Build history of the part. All positions in model axes, mm. A direction names the side the tool comes from. Coordinates: 2 decimals unless noted, no trailing zeros. Loops run counter-clockwise (first coordinate to the right, second up) from the corner with the lowest first, then second, coordinate; pieces in that order, holes last.
Item 1: Cut at C-C (x = -2.5). List the corners of the cut face in (y, z), and give its area (3 significant figures).
Item 2: 3-axis set-ups, long thin cutter, end or side, ignore diameter. For faces 1 (the face through (27.59, 1.05, 3.91)), 2 (the face through (0, -7.6, 11)), 3 (the face through (0, 7.6, 11)), 4 (the face through (0, 18, 2)), 5 (the face through (-10.336, -11.567, 1.724)): which of +Z, -Z, +X, -X, +Y, -Y reach the whole face in a straight line?
Item 3: Mould opens along X. For faces 6 (the face through (18.85, 0.17, 10.63)), 7 (the face through (0, -18, 2)), 8 (the face through (-29.246, -0.396, 2.169)), 9 (the face through (12.87, 13.51, 1.72)) say: released by +X, released by -X, zero draft, split by the parting line, or undercut.
Item 4: Drill centre lines: line 1 along Y through (x, z) = (11.25, 1.6); line 2 along X through (y, z) = (2, 5.5); line 3 along Z through (x, y) = (-19.5, 6). Where is each one in solid material? Low to high.
Item 5: Cut at A-A (z = 14). List the corners of the cut face in (x, y), and give its area (3 significant figures).
Item 6: Cut at D-D (y = -13). List the corners of the cut face in (x, z), and give its area (3 significant figures).
Item 7: Flat gauge pins, fed straight in: pin 1 (1 mm diameter, centred on x = -16, z = 14, fed in from -Y); pin 2 (8 mm diameter, centred on x = 4.5, y = -8, fed in from -Z); pin 3 (5.5 mm diameter, centred on x = 22.5, y = 0.5, fed in from +Z); pin 4 (8 mm diameter, centred on y = -8, z = 3.5, fed in from +X). Where does each tip first touch, or does it go through?
Item 8: Cut at B-B (x = 24.25). List the corners of the cut face in (y, z), and give its area (3 significant figures).
from build123d import *

# Parameters (mm, degrees)
OVAL_BASE_FLANGE_DEPTH       = 4.4
RAISED_OBROUND_HOUSING_DEPTH = 11.6
HOUSING_SLOT_R5_DEPTH        = 5
MOUNTING_HOLES_SKETCH_R      = 1.7
MOUNTING_HOLES_6X_3_4_DEPTH  = 5
COUNTERBORE_SKETCH_R         = 3.5
COUNTERBORES_6X_7_DEPTH      = 1
SLOT_THROUGH_CUT_SKETCH_R    = 2.5
SLOT_THROUGH_CUT_DEPTH       = 37.063312383
HOUSING_BASE_FILLET_R1_R     = 1


with BuildPart() as part:
    # Flange Profile Sketch → Oval Base Flange (new body)
    with BuildSketch(Plane.XY):
        with BuildLine():
            Line((-11.25, 18), (11.25, 18))
            ThreePointArc((11.25, 18), (29.25, 0), (11.25, -18))
            Line((11.25, -18), (-11.25, -18))
            ThreePointArc((-11.25, -18), (-29.25, 0), (-11.25, 18))
        make_face()
    extrude(amount=OVAL_BASE_FLANGE_DEPTH)

    # Housing Profile Sketch → Raised Obround Housing (add)
    with BuildSketch(Plane.XY.offset(4.4)):
        with BuildLine():
            Line((-11.25, 7.6), (11.25, 7.6))
            ThreePointArc((11.25, 7.6), (18.85, 0), (11.25, -7.6))
            Line((11.25, -7.6), (-11.25, -7.6))
            ThreePointArc((-11.25, -7.6), (-18.85, 0), (-11.25, 7.6))
        make_face()
    extrude(amount=RAISED_OBROUND_HOUSING_DEPTH)

    # Housing Slot Sketch → Housing Slot R5 (cut)
    with BuildSketch(Plane.XY.offset(16)):
        with BuildLine():
            Line((-11.25, 5), (11.25, 5))
            ThreePointArc((11.25, 5), (16.25, 0), (11.25, -5))
            Line((11.25, -5), (-11.25, -5))
            ThreePointArc((-11.25, -5), (-16.25, 0), (-11.25, 5))
        make_face()
    extrude(amount=-HOUSING_SLOT_R5_DEPTH, mode=Mode.SUBTRACT)

    # Mounting Holes Sketch → Mounting Holes 6xØ3.4 (cut)
    with BuildSketch(Plane.XY.offset(4.4)):
        with Locations((-24.22204296, 0)):
            Circle(MOUNTING_HOLES_SKETCH_R)
        with Locations((-11.25, 13)):
            Circle(MOUNTING_HOLES_SKETCH_R)
        with Locations((11.25, 13)):
            Circle(MOUNTING_HOLES_SKETCH_R)
        with Locations((24.25, 0)):
            Circle(MOUNTING_HOLES_SKETCH_R)
        with Locations((11.25, -13)):
            Circle(MOUNTING_HOLES_SKETCH_R)
        with Locations((-11.25, -13)):
            Circle(MOUNTING_HOLES_SKETCH_R)
    extrude(amount=-MOUNTING_HOLES_6X_3_4_DEPTH, mode=Mode.SUBTRACT)

    # Counterbore Sketch → Counterbores 6xØ7 (cut)
    with BuildSketch(Plane.XY.offset(4.4)):
        with Locations((-24.22204296, 0)):
            Circle(COUNTERBORE_SKETCH_R)
        with Locations((-11.25, 13)):
            Circle(COUNTERBORE_SKETCH_R)
        with Locations((11.25, 13)):
            Circle(COUNTERBORE_SKETCH_R)
        with Locations((24.25, 0)):
            Circle(COUNTERBORE_SKETCH_R)
        with Locations((11.25, -13)):
            Circle(COUNTERBORE_SKETCH_R)
        with Locations((-11.25, -13)):
            Circle(COUNTERBORE_SKETCH_R)
    extrude(amount=-COUNTERBORES_6X_7_DEPTH, mode=Mode.SUBTRACT)

    # Slot Through Cut Sketch → Slot Through Cut (cut, through all)
    with BuildSketch(Plane.XY.offset(11)):
        with Locations((-11.25, 0)):
            Circle(SLOT_THROUGH_CUT_SKETCH_R)
        with Locations((11.25, 0)):
            Circle(SLOT_THROUGH_CUT_SKETCH_R)
    extrude(amount=-SLOT_THROUGH_CUT_DEPTH, mode=Mode.SUBTRACT)

    # Housing Base Fillet R1
    housing_base_fillet_r1_edges = [part.edges().sort_by_distance(p)[0] for p in [
        (-18.85, 0, 4.4),
        (0, -7.6, 4.4),
        (18.85, 0, 4.4),
        (0, 7.6, 4.4),
    ]]
    fillet(housing_base_fillet_r1_edges, radius=HOUSING_BASE_FILLET_R1_R)


solid = part.part
Filled sheet:
1. outline: (-18, 0) - (18, 0) - (18, 4.4) - (8.6, 4.4) arc R1 cw to (7.6, 5.4) - (7.6, 16) - (5, 16) - (5, 11) - (-5, 11) - (-5, 16) - (-7.6, 16) - (-7.6, 5.4) arc R1 cw to (-8.6, 4.4) - (-18, 4.4) - close
1. area: 285 mm2
2. face 1: +Z
2. face 2: +Z, +X, -X, -Y
2. face 3: +Z, +X, -X, +Y
2. face 4: +Z, -Z, +X, -X, +Y
2. face 5: +Z, -Z
3. face 6: released by +X
3. face 7: zero draft
3. face 8: released by -X
3. face 9: undercut
4. line 1: y = -18 to -14.7, -11.3 to -2.5, 2.5 to 11.3, 14.7 to 18
4. line 2: x = -18.58 to -12.75, -9.75 to 9.75, 12.75 to 18.58
4. line 3: z = 0 to 4.4
5. outline: (-11.25, -7.6) - (11.25, -7.6) arc R7.6 ccw to (11.25, 7.6) - (-11.25, 7.6) arc R7.6 ccw to start; hole (-11.25, -5) - (11.25, -5) arc R5 ccw to (11.25, 5) - (-11.25, 5) arc R5 ccw to start
5. area: 220 mm2
6. outline: (-23.7, 0) - (-12.95, 0) - (-12.95, 3.4) - (-14.75, 3.4) - (-14.75, 4.4) - (-23.7, 4.4) - close; (-9.55, 0) - (9.55, 0) - (9.55, 3.4) - (7.75, 3.4) - (7.75, 4.4) - (-7.75, 4.4) - (-7.75, 3.4) - (-9.55, 3.4) - close; (12.95, 0) - (23.7, 0) - (23.7, 4.4) - (14.75, 4.4) - (14.75, 3.4) - (12.95, 3.4) - close
6. area: 171 mm2
7. pin 1: stops at y = -6.3
7. pin 2: stops at z = 0
7. pin 3: stops at z = 4.4
7. pin 4: stops at x = 28.8
8. outline: (-12.45, 0) - (-1.7, 0) - (-1.7, 3.4) - (-3.5, 3.4) - (-3.5, 4.4) - (-12.45, 4.4) - close; (1.7, 0) - (12.45, 0) - (12.45, 4.4) - (3.5, 4.4) - (3.5, 3.4) - (1.7, 3.4) - close
8. area: 91.0 mm2
